Here's the drawing with two shaded views (mm, measured from the low corner). I have some questions. A direction names the side the tool comes from. Round coordinates to 2 decimals unless told otherwise and drop trailing zeros. Loops run counter-clockwise (first coordinate to the right, second up) from the corner with the lowest first, then second, coordinate; pieces in that order, holes last. Notation, with made-up numbers: (89, 49.25) -> (101, 49.25) arc R9 cw to (101, 64.25) -> close; hole circle Ø3 at (61.5, -1). An arc over 180 degrees is marked (long way). Write each question's results on one line, items separated by ' | '.
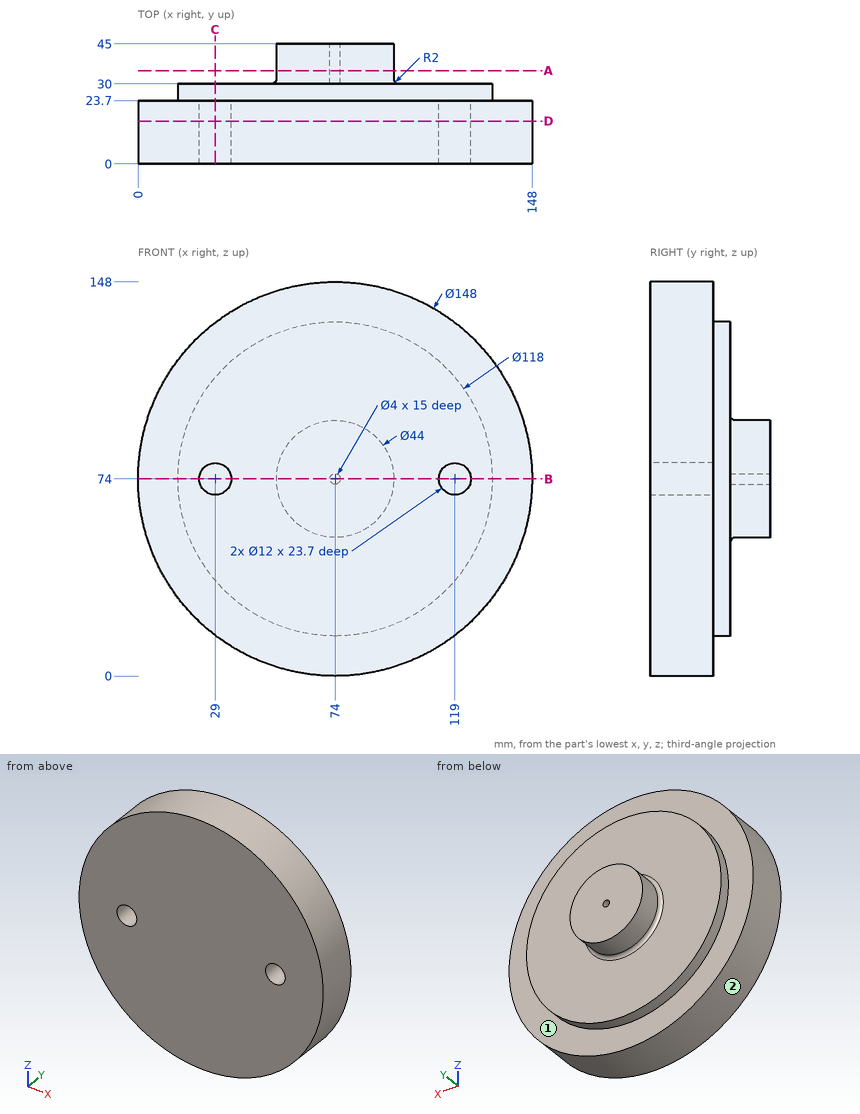
1. If we section it at C-C (x = 29): List the corners of the cut face in (y, z) for me.
Final values:
outline: (0, 15.25) -> (23.7, 15.25) -> (23.7, 35.84) -> (30, 35.84) -> (30, 112.16) -> (23.7, 112.16) -> (23.7, 132.75) -> (0, 132.75) -> (0, 80) -> (23.7, 80) -> (23.7, 68) -> (0, 68) -> close
2. If we section it at A-A (y = 35): List the corners of the cut face in (x, z) for me, then the cut area to 3 significant figures.
Final values:
outline: circle Ø44 at (74, 74); hole circle Ø4 at (74, 74) | area: 1,510 mm2
3. On a 3-axis mill with a long thin cutter (end or side, diameter ignored), from which of +Z, -Z, +X, -X, +Y, -Y can I reach the whole of each face in a straight line? I mean the marked faces 1 and 2. Say none if no direction works.
Final values:
face 1: +Y | face 2: +Y, -Y
4. Please list where these lines run through material, in increasing order: line 1 (X direction, y = 18, z = 74); line 2 (Z direction, x = 74, y = 36.5); line 3 (Y direction, x = 56.5, z = 56.5). Write a range as from..to.
Final values:
line 1: 0..23, 35..113, 125..148 | line 2: 52..72, 76..96 | line 3: 0..30
5. If we section it at D-D (y = 16): List the corners of the cut face in (x, z) for me, then the cut area to 3 significant figures.
Final values:
outline: circle Ø148 at (74, 74); hole circle Ø12 at (29, 74); hole circle Ø12 at (119, 74) | area: 17,000 mm2
6. If we section it at B-B (z = 74): List the corners of the cut face in (x, y) for me, then the cut area to 3 significant figures.
Final values:
outline: (0, 0) -> (23, 0) -> (23, 23.7) -> (35, 23.7) -> (35, 0) -> (113, 0) -> (113, 23.7) -> (125, 23.7) -> (125, 0) -> (148, 0) -> (148, 23.7) -> (133, 23.7) -> (133, 30) -> (98, 30) arc R2 cw to (96, 32) -> (96, 45) -> (76, 45) -> (76, 30) -> (72, 30) -> (72, 45) -> (52, 45) -> (52, 32) arc R2 cw to (50, 30) -> (15, 30) -> (15, 23.7) -> (0, 23.7) -> close | area: 4,280 mm2
7. Will these pins go through, and if not, where does the flat tip stop? pin 1 (3.5 mm diameter, centred on x = 121, z = 76.5, fed in from -Y); pin 2 (4 mm diameter, centred on x = 114.5, y = 23, fed in from -Z); pin 3 (3 mm diameter, centred on x = 87.5, y = 29, fed in from +Z).
Final values:
pin 1: y = 23.7 | pin 2: z = 10.8 | pin 3: z = 131.77
